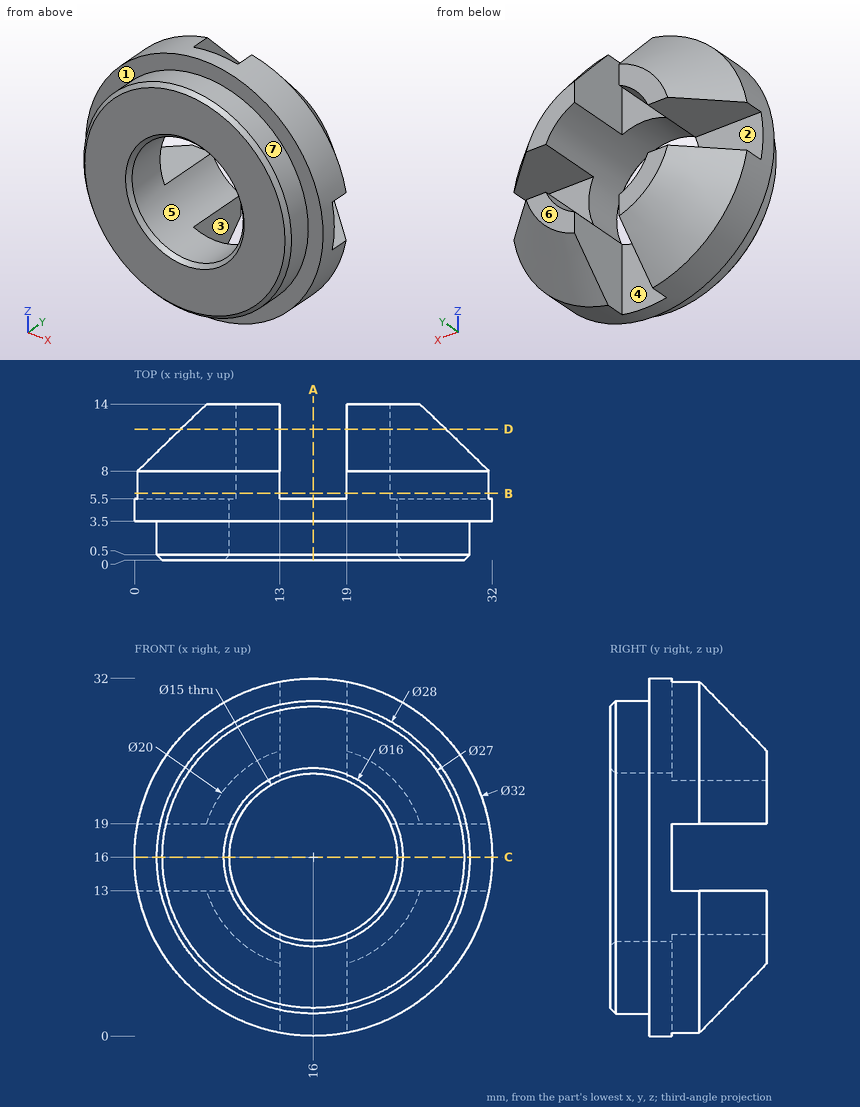
Check sheet for the drawn part. Datum: minimum x, y, z corner. Units: mm. A direction names the side the tool comes from. Round coordinates to 2 decimals unless told otherwise and drop trailing zeros. Loops run counter-clockwise (first coordinate to the right, second up) from the corner with the lowest first, then second, coordinate; pieces in that order, holes last. Notation, with made-up numbers: (58, 4) - (64, 4) arc R16 cw to (64, 14) - close; hole circle Ø7 at (-20.75, 12). An arc over 180 degrees is marked (long way). Answer as a JSON object with one key per item and string values. Group by question number.
Q1. Sectioned sample at C-C, the plane z = 16. Enter the section's corners in (x, y).
Q2. Sectioned sample at D-D, the plane y = 11.75. Enter the section's corners in (x, z), plus the area to 3 significant figures.
Q3. Sectioned sample at A-A, the plane x = 16. Enter the section's corners in (y, z).
Q4. Gauge pin test, flat ends, axial feed: P1, Ø1.5, axis at x = 11.5, z = 4.5, coming from the +Y side; P2, Ø7, axis at y = 10, z = 3, coming from the -X side; P3, Ø3, axis at x = 29, z = 16.5, coming from the +Y side; P4, Ø8, axis at x = 25.5, z = 16, coming from the +Y side. Record the tip position at first contact, or that the pin passes through.
Q5. Scan lines: line 1 along X through (y, z) = (4.75, 16); line 2 along Y through (x, z) = (24, 16.5); line 3 along X through (y, z) = (1.5, 18). Record each from-to range of solid material in increasing order. Write a range as [from, to].
Q6. Mould release check, pull along X, two halves, no side actions. Record for the marked faces 4, 5, 6 and 7: released by +X, released by -X, zero draft, split by the parting line, or undercut.
Q7. Set-up check for the marked faces 1, 2 and 3: record each of +Z, -Z, +X, -X, +Y, -Y from which the full face is reachable in a straight line by a thin tool's end or side.
Q8. Sectioned sample at B-B, the plane y = 6. Enter the section's corners in (x, z).
Solution:
{
 "1": {"outline": "(0, 3.5) - (2, 3.5) - (2, 0.5) - (2.5, 0) - (8, 0) - (8.5, 0.5) - (8.5, 5.5) - (0, 5.5) - close; (23.5, 0.5) - (24, 0) - (29.5, 0) - (30, 0.5) - (30, 3.5) - (32, 3.5) - (32, 5.5) - (23.5, 5.5) - close"},
 "2": {"outline": "(4.12, 13) arc R12.25 ccw to (13, 4.12) - (13, 9.13) arc R7.5 cw to (9.13, 13) - close; (4.12, 19) - (9.13, 19) arc R7.5 cw to (13, 22.87) - (13, 27.88) arc R12.25 ccw to start; (19, 4.12) arc R12.25 ccw to (27.88, 13) - (22.87, 13) arc R7.5 cw to (19, 9.13) - close; (19, 22.87) arc R7.5 cw to (22.87, 19) - (27.88, 19) arc R12.25 ccw to (19, 27.88) - close", "area": "179 mm²"},
 "3": {"outline": "(0, 2.5) - (0.5, 2) - (3.5, 2) - (3.5, 0) - (5.5, 0) - (5.5, 8.5) - (0.5, 8.5) - (0, 8) - close; (0, 24) - (0.5, 23.5) - (5.5, 23.5) - (5.5, 32) - (3.5, 32) - (3.5, 30) - (0.5, 30) - (0, 29.5) - close"},
 "4": {"P1": "stops at y = 12.4", "P2": "stops at x = 3.61", "P3": "stops at y = 5.5", "P4": "stops at y = 14"},
 "5": {"line 1": "x = [0, 8.5], [23.5, 32]", "line 2": "y = [0, 5.5]", "line 3": "x = [2.14, 8.77], [23.23, 29.86]"},
 "6": {"face 4": "undercut", "face 5": "undercut", "face 6": "zero draft", "face 7": "split by the parting line"},
 "7": {"face 1": "-Y", "face 2": "+X, -X, +Y", "face 3": "+Z, -Z, +Y"},
 "8": {"outline": "(0.28, 13) arc R16 ccw to (13, 0.28) - (13, 9.13) arc R7.5 cw to (9.13, 13) - close; (0.28, 19) - (9.13, 19) arc R7.5 cw to (13, 22.87) - (13, 31.72) arc R16 ccw to start; (19, 0.28) arc R16 ccw to (31.72, 13) - (22.87, 13) arc R7.5 cw to (19, 9.13) - close; (19, 22.87) arc R7.5 cw to (22.87, 19) - (31.72, 19) arc R16 ccw to (19, 31.72) - close"}
}
